from build123d import *

# Parameters (mm, degrees)
BOSS_EXTRUDE1_DEPTH     = 22.4
CUT_EXTRUDE1_DEPTH      = 7
CUT_EXTRUDE1_DEPTH_BACK = 7
CUT_EXTRUDE2_DEPTH      = 19.8
CUT_EXTRUDE3_DEPTH      = 2.5
CUT_EXTRUDE4_DEPTH      = 5.925
CUT_EXTRUDE4_DEPTH_BACK = 5.925
CUT_EXTRUDE5_DEPTH      = 7
CUT_EXTRUDE5_DEPTH_BACK = 7
CUT_EXTRUDE6_DEPTH      = 26.1
CUT_EXTRUDE6_DEPTH_BACK = 26.1


with BuildPart() as part:
    # Sketch1 → Boss-Extrude1 (new body)
    with BuildSketch(Plane.XY):
        with BuildLine():
            Line((-7, 21.1), (-7, 0))
            Line((-7, 0), (7, 0))
            Line((7, 0), (7, 21.1))
            ThreePointArc((7, 21.1), (5.535533906, 24.635533906), (2, 26.1))
            Line((2, 26.1), (-2, 26.1))
            ThreePointArc((-2, 26.1), (-5.535533906, 24.635533906), (-7, 21.1))
        make_face()
    extrude(amount=BOSS_EXTRUDE1_DEPTH)

    # Sketch2 → Cut-Extrude1 (cut, two sides: drawn at the far end of the back side and taken through both)
    with BuildSketch(Plane(origin=(0, 0, 0), x_dir=(0, 0, -1), z_dir=(1, 0, 0)).offset(-CUT_EXTRUDE1_DEPTH_BACK)):
        Polygon((-7.9, 2), (-7.9, 0), (-6.745299462, 0), align=None)
    extrude(amount=CUT_EXTRUDE1_DEPTH + CUT_EXTRUDE1_DEPTH_BACK, mode=Mode.SUBTRACT)

    # Sketch4 → Cut-Extrude2 (cut)
    with BuildSketch(Plane.XY.offset(7.9)):
        with BuildLine():
            Line((-7, 26.1), (-7, 0))
            Line((-7, 0), (9, 0))
            Line((9, 0), (9, 16.5))
            Line((9, 16.5), (7, 16.5))
            ThreePointArc((7, 16.5), (5.535533906, 12.964466094), (2, 11.5))
            Line((2, 11.5), (-3, 11.5))
            Line((-3, 11.5), (-3, 26.1))
            Line((-3, 26.1), (-7, 26.1))
        make_face()
    extrude(amount=CUT_EXTRUDE2_DEPTH, mode=Mode.SUBTRACT)

    # Sketch3 → Cut-Revolve1 (revolve, cut)
    with BuildSketch(Plane(origin=(0, 0, 0), x_dir=(0, 0, -1), z_dir=(1, 0, 0)), mode=Mode.PRIVATE) as cut_revolve1_sk:
        Polygon((-0.7, 6.7), (-0.7, 10.45), (-1.2, 10.95), (-5.7, 10.95), (-5.7, 11.7), (0, 11.7), (0, 6.7), align=None)
    revolve(cut_revolve1_sk.sketch.rotate(Axis((0, 6.7, 0), (0, 0, 1)), 270), axis=Axis((0, 6.7, 0), (0, 0, 1)), mode=Mode.SUBTRACT)

    # Sketch5 → Cut-Extrude3 (cut)
    with BuildSketch(Plane(origin=(0, 0, 0.7), x_dir=(-1, 0, 0), z_dir=(0, 0, -1))):
        Polygon((1.154700538, 4.7), (2.309401077, 6.7), (1.154700538, 8.7), (-1.154700538, 8.7), (-2.309401077, 6.7), (-1.154700538, 4.7), align=None)
    extrude(amount=-CUT_EXTRUDE3_DEPTH, mode=Mode.SUBTRACT)

    # Sketch6 → Cut-Extrude4 (cut, two sides: drawn at the far end of the back side and taken through both)
    with BuildSketch(Plane.XY.offset(5.925).offset(-CUT_EXTRUDE4_DEPTH_BACK)):
        with BuildLine():
            Line((-7, 14.2), (-5, 14.2))
            ThreePointArc((-5, 14.2), (-3.585786438, 14.785786438), (-3, 16.2))
            Line((-3, 16.2), (-3, 26.1))
            Line((-3, 26.1), (-7, 26.1))
            Line((-7, 26.1), (-7, 14.2))
        make_face()
    extrude(amount=CUT_EXTRUDE4_DEPTH + CUT_EXTRUDE4_DEPTH_BACK, mode=Mode.SUBTRACT)

    # Sketch7 → Cut-Extrude5 (cut, two sides: drawn at the far end of the back side and taken through both)
    with BuildSketch(Plane(origin=(0, 0, 0), x_dir=(0, 0, -1), z_dir=(1, 0, 0)).offset(-CUT_EXTRUDE5_DEPTH_BACK)):
        with BuildLine():
            Line((-11.419615242, 11.4), (-7.9, 11.4))
            Line((-7.9, 11.4), (-7.9, 11.7))
            ThreePointArc((-7.9, 11.7), (-8.4, 12.566025404), (-9.4, 12.566025404))
            Line((-9.4, 12.566025404), (-11.419615242, 11.4))
        make_face()
    extrude(amount=CUT_EXTRUDE5_DEPTH + CUT_EXTRUDE5_DEPTH_BACK, mode=Mode.SUBTRACT)

    # Sketch8 → Cut-Extrude6 (cut, two sides: drawn at the far end of the back side and taken through both)
    with BuildSketch(Plane(origin=(0, 0, 0), x_dir=(1, 0, 0), z_dir=(0, 1, 0)).offset(-CUT_EXTRUDE6_DEPTH_BACK)):
        Polygon((3.016283143, -22.4), (7, -22.4), (7, -20.1), align=None)
    extrude(amount=CUT_EXTRUDE6_DEPTH + CUT_EXTRUDE6_DEPTH_BACK, mode=Mode.SUBTRACT)

    # Sketch9 → Revolve1 (revolve)
    with BuildSketch(Plane(origin=(0, 0, 0), x_dir=(0, 0, -1), z_dir=(1, 0, 0)), mode=Mode.PRIVATE) as revolve1_sk:
        Polygon((-13.7, 6.7), (-13.7, 8.7095), (-13.2095, 9.2), (-7.9, 9.2), (-7.9, 6.7), align=None)
    revolve(revolve1_sk.sketch.rotate(Axis((0, 6.7, 7.9), (0, 0, 1)), 270), axis=Axis((0, 6.7, 7.9), (0, 0, 1)))


solid = part.part
Part model, mm, in its own coordinate system. A direction names the side the tool comes from. Round coordinates to 2 decimals unless told otherwise and drop trailing zeros. Write each loop counter-clockwise with the first axis right and the second up, starting at its lowest first coordinate (ties: lowest second). Pieces come first, ordered by that corner, then holes. Notation, with made-up numbers: M 56,75.5 L 106,75.5 A13 ccw 106,89.5 Z; hole C 72,69 d4. An arc over 180 degrees is marked long. Return JSON: item names as keys, results as strings. Group by question number.
(1) Which spindle directions (+Z, -Z, +X, -X, +Y, -Y) get a long thin tool onto all of the face, cutting with end or side? Do faces 1 (the face through (1.724, 7.714, 1.932)), 2 (the face through (-0.54, 4.26, 10.52)), 3 (the face through (0, 7, 13.7)). Say none if no direction does.
(2) Saw through at D-D on x = -5.5. Write the cut outline in (y, z), then the cut area to 3 significant figures.
(3) Pin check, flat tips, straight feed: pin 1 Ø4 at (x, z) = (0.5, 18) entering from -Y; pin 2 Ø6 at (x, y) = (0, 6.7) entering from -Z; pin 3 Ø2 at (y, z) = (3.5, 10) entering from -X. Stop position of each tip, or through.
(4) Two-plate mould, pull along X, no slides. Class faces 4 (the face through (-0.553, 10.914, 3.481)), 5 (the face through (7, 13, 5)), 6 (the face through (-0.098, 0.986, 7.315)): +X half, -X half, draft (parallel to the pull), parting line (faces both ways), or undercut.
(5) Saw through at C-C on z = 19. Write the cut outline in (x, y).
(6) Saw through at A-A on z = 10.75. Write the cut outline in (x, y).
(7) Drill centre lines: probe 1 along Y at (x, z) = (0, 3.1); probe 2 along Y at (x, z) = (0, 3.4); probe 3 along Y at (x, z) = (1.5, 1.25). Where is each one in solid material? Low to high.
Returned:
{
 "1": {"face 1": "-Z", "face 2": "+Z", "face 3": "+Z, +X, -X, -Y"},
 "2": {"outline": "M 0,0 L 14.2,0 L 14.2,7.9 L 2,7.9 L 0,6.75 Z", "area": "111 mm²"},
 "3": {"pin 1": "y = 11.5", "pin 2": "z = 0.7", "pin 3": "x = -1.19"},
 "4": {"face 4": "undercut", "face 5": "+X half", "face 6": "draft"},
 "5": {"outline": "M -3,11.5 L 2,11.5 A5 ccw 7,16.5 L 7,21.1 A5 ccw 2,26.1 L -2,26.1 A5 ccw -3,26 Z"},
 "6": {"outline": "M -3,11.79 L 3.67,11.79 A5 ccw 7,16.5 L 7,21.1 A5 ccw 2,26.1 L -2,26.1 A5 ccw -3,26 Z; C 0,6.7 d5"},
 "7": {"probe 1": "0 to 1.7, 2.45 to 4.7, 8.7 to 10.95, 11.7 to 26.1", "probe 2": "0 to 1.7, 2.45 to 10.95, 11.7 to 26.1", "probe 3": "0 to 1.93, 2.72 to 5.3, 8.1 to 10.68, 11.47 to 26.1"}
}
